from build123d import *

# Parameters (mm, degrees)
SKETCH1_W                                   = 25
SKETCH1_H                                   = 75
EXTRUDE_THIN1_DEPTH                         = 6
CHAMFER1_SIZE                               = 1
HOLE_SIZE_PER_SOCKET_FLAT_COUNTEBLZ_2_COUNT = 2
HOLE_SIZE_PER_SOCKET_FLAT_COUNTEBLZ_2_PITCH = 59
CHAMFER2_SIZE                               = 10
M6_TAPPED_HOLE1_D                           = 5
SKETCH12_W                                  = 20.259222761
SKETCH12_H                                  = 26
CUT_EXTRUDE1_DEPTH                          = 10
CHAMFER3_SIZE                               = 1


with BuildPart() as part:
    # Sketch1 → Extrude-Thin1 (new body)
    with BuildSketch(Plane.XY):
        with Locations((-12.5, 37.5)):
            Rectangle(SKETCH1_W, SKETCH1_H)
    extrude(amount=EXTRUDE_THIN1_DEPTH)

    # Chamfer1
    chamfer1_edges = [part.edges().sort_by_distance(p)[0] for p in [
        (0, 75, 3),
        (0, 0, 3),
    ]]
    chamfer(chamfer1_edges, length=CHAMFER1_SIZE)

    # Sketch9 → Hole size (per socket flat counteBLZKk head screw type)1 (revolve, cut)
    with BuildSketch(Plane(origin=(-7.5, 67, 6), x_dir=(0, -1, 0), z_dir=(1, 0, 0))):
        Polygon((0, 0), (0, 6), (3.3, 6), (3.3, 3.2), (6.5, 0), align=None)
    hole_size_per_socket_flat_counteblzkk_h = revolve(axis=Axis((-7.5, 67, 12.35), (0, 0, -1)), mode=Mode.SUBTRACT)

    # Hole size _per socket flat counteBLZ 2: Hole size (per socket flat counteBLZKk head screw type)1 ×2
    with Locations(*[(0, -i * HOLE_SIZE_PER_SOCKET_FLAT_COUNTEBLZ_2_PITCH, 0) for i in range(1, HOLE_SIZE_PER_SOCKET_FLAT_COUNTEBLZ_2_COUNT)]):
        add(hole_size_per_socket_flat_counteblzkk_h, mode=Mode.SUBTRACT)

    # Chamfer2
    chamfer2_edges = [part.edges().sort_by_distance(p)[0] for p in [
        (-25, 75, 3),
        (-25, 0, 3),
    ]]
    chamfer(chamfer2_edges, length=CHAMFER2_SIZE)

    # M6 Tapped Hole1 (through all)
    with Locations(Plane.XY.offset(6)):
        with Locations((-18, 37.5)):
            Hole(M6_TAPPED_HOLE1_D / 2)

    # Sketch12 → Cut-Extrude1 (cut)
    with BuildSketch(Plane.XY.offset(6)):
        with Locations((5.129611381, 37.5)):
            Rectangle(SKETCH12_W, SKETCH12_H)
    extrude(amount=-CUT_EXTRUDE1_DEPTH, mode=Mode.SUBTRACT)

    # Chamfer3
    chamfer3_edges = [part.edges().sort_by_distance(p)[0] for p in [
        (0, 50.5, 3),
        (0, 24.5, 3),
    ]]
    chamfer(chamfer3_edges, length=CHAMFER3_SIZE)


solid = part.part
The listing builds one solid part. Answer for the finished solid, in the listing's coordinates (mm). A direction names the side the tool comes from. Give positions to 0.01 mm unless a question says otherwise; leave off trailing zeros. Write each loop counter-clockwise with the first axis right and the second up, starting at its lowest first coordinate (ties: lowest second). Pieces come first, ordered by that corner, then holes.
1) Section D-D (x = -7.5) is taken. Write down the section's boundary in (y, z), and give its area (3 significant figures).
2) A tool of negligible diameter and unlimited length cuts with its end or side. For faces 1 (the face through (-7.6, 70.3, 1.4)), 2 (the face through (-3, 24.5, 3)), from which of +Z, -Z, +X, -X, +Y, -Y can it reach the whole face along a straight path? Write none if from no direction.
3) Section A-A (y = 37.5) is taken. Write down the section's boundary in (x, z).
4) Given P1, Ø8.5, axis at x = -7.5, y = 8, coming from the +Z side; P2, Ø8, axis at x = -18, y = 37.5, coming from the +Z side; P3, Ø1.8, axis at y = 33, z = 4.5, coming from the +X side; P4, Ø5.5, axis at x = -7.5, y = 67, coming from the -Z side, each flat-ended and moving along its own axis, determine where each tip first touches the part or whether it passes through.
5) Section B-B (z = 4.4) is taken. Write down the section's boundary in (x, y).
6) For a pull along X with two mould halves and no side action, classify faces 3 (the face through (0, 63, 3)), 4 (the face through (-25, 37, 3)), 5 (the face through (-7.6, 11.3, 1.4)) as pulls with the +X half, pulls with the -X half, needs draft (parallel to the pull), parting line crosses it, or undercut.
7) Section C-C (x = -18) is taken. Write down the section's boundary in (y, z).
8) Find the intervals of material crossed by L1, parallel to Y at x = -7.5, z = 1.2; L2, parallel to Y at x = -2.75, z = 0.6; L3, parallel to Y at x = -5.5, z = 4.9, in increasing order.
Response:
1. outline: (0, 0) - (4.7, 0) - (4.7, 2.8) - (1.5, 6) - (0, 6) - close; (11.3, 0) - (63.7, 0) - (63.7, 2.8) - (60.5, 6) - (14.5, 6) - (11.3, 2.8) - close; (70.3, 0) - (75, 0) - (75, 6) - (73.5, 6) - (70.3, 2.8) - close
1. area: 350 mm2
2. face 1: +Z, -Z
2. face 2: +Z, -Z, +X
3. outline: (-25, 0) - (-20.5, 0) - (-20.5, 6) - (-25, 6) - close; (-15.5, 0) - (-5, 0) - (-5, 6) - (-15.5, 6) - close
4. P1: stops at z = 3.75
4. P2: stops at z = 6
4. P3: stops at x = -5
4. P4: passes through
5. outline: (-25, 10) - (-15, 0) - (-1, 0) - (0, 1) - (0, 23.5) - (-1, 24.5) - (-5, 24.5) - (-5, 50.5) - (-1, 50.5) - (0, 51.5) - (0, 74) - (-1, 75) - (-15, 75) - (-25, 65) - close; hole circle Ø5 at (-18, 37.5); hole circle Ø9.8 at (-7.5, 8); hole circle Ø9.8 at (-7.5, 67)
6. face 3: pulls with the +X half
6. face 4: pulls with the -X half
6. face 5: undercut
7. outline: (3, 0) - (35, 0) - (35, 6) - (3, 6) - close; (40, 0) - (72, 0) - (72, 6) - (40, 6) - close
8. L1: y = 0 to 4.7, 11.3 to 63.7, 70.3 to 75
8. L2: y = 0 to 24.5, 50.5 to 75
8. L3: y = 0 to 2.98, 13.02 to 61.98, 72.02 to 75
